Could you check a few things on this model? Use its own coordinates, in mm. A direction names the side the tool comes from. Give positions to 0.01 mm unless a question says otherwise; leave off trailing zeros. Write each loop counter-clockwise with the first axis right and the second up, starting at its lowest first coordinate (ties: lowest second). Pieces come first, ordered by that corner, then holes. Notation, with made-up numbers: (38.25, 63) - (88.25, 63) arc R25 cw to (88.25, 84) - close; hole circle Ø4 at (-38.5, 54.5). An arc over 180 degrees is marked (long way). Use one line per item in the form item = value.
```python
from build123d import *

# Parameters (mm, degrees)
BOSS_EXTRUDE1_DEPTH = 3


with BuildPart() as part:
    # Sketch1 → Boss-Extrude1 (new, symmetric)
    with BuildSketch(Plane.XY):
        Polygon((43.6, -110), (-156.4, -110), (-156.4, -100), (-161.9, -100), (-161.9, -75), (-156.4, -75), (-156.4, -65), (43.6, -65), (43.6, -75), (49.1, -75), (49.1, -100), (43.6, -100), align=None)
    extrude(amount=BOSS_EXTRUDE1_DEPTH, both=True)


solid = part.part
```
1. If I drill on line 1 (X direction, y = -71.5, z = 1.5), over which ranges is the centre line in solid material (lowest first)? Write a range as from..to.
Response values:
line_1 = -156.4..43.6
2. Imagine slicing it at A-A, the plane z = -0.75. List the corners of the cut face in (x, y) for me, and give its area (4 significant figures).
Response values:
outline = (-161.9, -100) - (-156.4, -100) - (-156.4, -110) - (43.6, -110) - (43.6, -100) - (49.1, -100) - (49.1, -75) - (43.6, -75) - (43.6, -65) - (-156.4, -65) - (-156.4, -75) - (-161.9, -75) - close
area = 9,275 mm²
3. Imagine slicing it at B-B, the plane y = -103. List the corners of the cut face in (x, z) for me.
Response values:
outline = (-156.4, -3) - (43.6, -3) - (43.6, 3) - (-156.4, 3) - close
4. Which directions (+Z, -Z, +X, -X, +Y, -Y) give clear straight access to the entire face, cutting with the end or side of a thin tool? Please do faces 1 (the face through (-156.4, -70, 0)), 2 (the face through (46, -100, 0)), 3 (the face through (-156.4, -105, 0)), 4 (the face through (43.6, -70, 0)).
Response values:
face_1 = +Z, -Z, -X, +Y
face_2 = +Z, -Z, +X, -Y
face_3 = +Z, -Z, -X, -Y
face_4 = +Z, -Z, +X, +Y
5. For pin 1 (1.6 mm diameter, centred on x = 46, z = 0.5, fed in from +Y); pin 2 (3 mm diameter, centred on x = -159, z = 1, fed in from -Y); pin 3 (1.8 mm diameter, centred on y = -68, z = 0.5, fed in from +X), each with a flat end and sliding along its axis, tell me the tip position at first contact or that it passes through.
Response values:
pin_1 = -75
pin_2 = -100
pin_3 = 43.6
